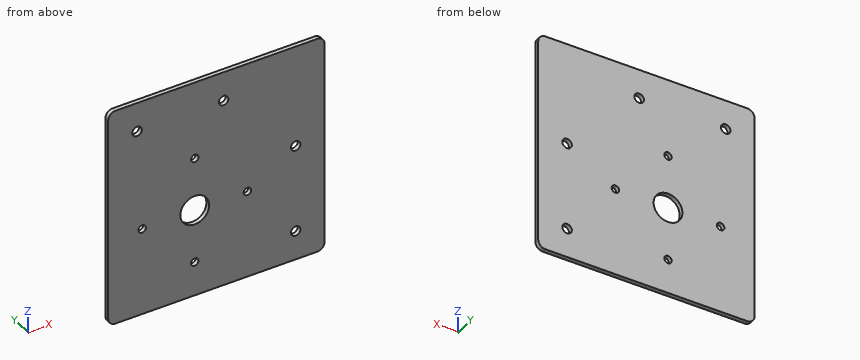
```python
from build123d import *

# Parameters (mm, degrees)
SKETCH_1_W              = 150
SKETCH_1_H              = 150
EXTRUDE_1_DEPTH         = 3
HOLE_WIZARD_6_6_6_6_1_D = 6.6
FILLET_1_R              = 5
SKETCH_4_R              = 10
SKETCH_4_R_2            = 2.6
CUT_EXTRUDE_1_DEPTH     = 107.108435103


with BuildPart() as part:
    # 草图1 → 凸台-拉伸1 (new body)
    with BuildSketch(Plane(origin=(0, 0, 0), x_dir=(1, 0, 0), z_dir=(0, 1, 0))):
        Rectangle(SKETCH_1_W, SKETCH_1_H)
    extrude(amount=EXTRUDE_1_DEPTH)

    # Ø6.6 (6.6) 直径孔1 (through all)
    with Locations(Plane(origin=(0, 3, 0), x_dir=(-1, 0, 0), z_dir=(0, 1, 0))):
        with Locations((-55, 5), (-5, 55), (55, 55), (-55, -55)):
            Hole(HOLE_WIZARD_6_6_6_6_1_D / 2)

    # 圆角1
    fillet_1_edges = [part.edges().sort_by_distance(p)[0] for p in [
        (75, 1.5, 75),
        (-75, 1.5, 75),
        (-75, 1.5, -75),
        (75, 1.5, -75),
    ]]
    fillet(fillet_1_edges, radius=FILLET_1_R)

    # 草图4 → 切除-拉伸1 (cut, through all)
    with BuildSketch(Plane(origin=(0, 3, 0), x_dir=(1, 0, 0), z_dir=(0, 1, 0))):
        with Locations(Location((-15, 15, 0), (0, 0, 270))):
            Circle(SKETCH_4_R)
        with Locations(Location((-15, 51.5, 0), (0, 0, 270))):
            Circle(SKETCH_4_R_2)
        with Locations(Location((21.5, 15, 0), (0, 0, 270))):
            Circle(SKETCH_4_R_2)
        with Locations(Location((-15, -21.5, 0), (0, 0, 270))):
            Circle(SKETCH_4_R_2)
        with Locations(Location((-51.5, 15, 0), (0, 0, 270))):
            Circle(SKETCH_4_R_2)
    extrude(amount=-CUT_EXTRUDE_1_DEPTH, mode=Mode.SUBTRACT)


solid = part.part
```
Here's how the part is built. I have some questions about the finished solid (model axes, mm). Give positions to 0.01 mm unless a question says otherwise; leave off trailing zeros. Write each loop counter-clockwise with the first axis right and the second up, starting at its lowest first coordinate (ties: lowest second). Pieces come first, ordered by that corner, then holes.
(1) Imagine slicing it at A-A, the plane y = 2.1. Count the separate pieces of the cut face and the enclosed holes in it, and give its area (3 significant figures).
Output values:
separate pieces: 1
enclosed holes: 9
area: 21,900 mm2
(2) If I drill on L1, parallel to X at y = 1.5, z = -51.5; L2, parallel to X at y = 2, z = -15; L3, parallel to Z at x = -55, y = 1.35, over which ranges is the centre line in solid material (lowest first)?
Output values:
L1: x = -75 to -17.6, -12.4 to 75
L2: x = -75 to -54.1, -48.9 to -25, -5 to 18.9, 24.1 to 75
L3: z = -75 to 51.7, 58.3 to 75
(3) Imagine slicing it at B-B, the plane z = -15. Write out the boundary of the cut face in (x, y).
Output values:
outline: (-75, 0) - (-54.1, 0) - (-54.1, 3) - (-75, 3) - close; (-48.9, 0) - (-25, 0) - (-25, 3) - (-48.9, 3) - close; (-5, 0) - (18.9, 0) - (18.9, 3) - (-5, 3) - close; (24.1, 0) - (75, 0) - (75, 3) - (24.1, 3) - close
(4) Imagine slicing it at D-D, the plane x = 55. Write out the boundary of the cut face in (y, z).
Output values:
outline: (0, -75) - (3, -75) - (3, -58.3) - (0, -58.3) - close; (0, -51.7) - (3, -51.7) - (3, 1.7) - (0, 1.7) - close; (0, 8.3) - (3, 8.3) - (3, 75) - (0, 75) - close
(5) Imagine slicing it at C-C, the plane x = 5. Write out the boundary of the cut face in (y, z), and give its area (3 significant figures).
Output values:
outline: (0, -75) - (3, -75) - (3, 51.7) - (0, 51.7) - close; (0, 58.3) - (3, 58.3) - (3, 75) - (0, 75) - close
area: 430 mm2
